from build123d import *
from OCP.BRepFilletAPI import BRepFilletAPI_MakeChamfer

# Parameters (mm, degrees)
BOSS_EXTRUDE1_DEPTH    = 694
SKETCH3_W              = 110
SKETCH3_H              = 70.171613021
CUT_EXTRUDE1_DEPTH     = 145
M10_TAPPED_HOLE2_D     = 8.5
M10_TAPPED_HOLE2_DEPTH = 24.5
M10_TAPPED_HOLE2_TIP   = 2.553657631
BOSS_EXTRUDE2_START    = 44
BOSS_EXTRUDE2_DEPTH    = 44
BOSS_EXTRUDE3_DEPTH    = 44
CUT_EXTRUDE3_DEPTH     = 100
CHAMFER1_SIZE          = 10
CHAMFER1_SIZE2         = 11.749570117
M6_TAPPED_HOLE1_D      = 5
M6_TAPPED_HOLE1_DEPTH  = 15
M6_TAPPED_HOLE1_TIP    = 1.502151548


with BuildPart() as part:
    # Sketch1 → Boss-Extrude1 (new body)
    with BuildSketch(Plane.XY):
        with BuildLine():
            Line((0, 0), (0, -100))
            Line((0, -100), (50, -100))
            Line((50, -100), (50, -98.925311188))
            ThreePointArc((50, -98.925311188), (48.896193111, -95.973045557), (46.126278954, -94.469104878))
            Line((46.126278954, -94.469104878), (13.317028642, -89.858065454))
            ThreePointArc((13.317028642, -89.858065454), (8.084968568, -87.017288616), (6, -81.440786869))
            Line((6, -81.440786869), (6, -18.559213131))
            ThreePointArc((6, -18.559213131), (8.084968568, -12.982711384), (13.317028642, -10.141934546))
            Line((13.317028642, -10.141934546), (46.126278954, -5.530895122))
            ThreePointArc((46.126278954, -5.530895122), (48.896193111, -4.026954443), (50, -1.074688812))
            Line((50, -1.074688812), (50, 0))
            Line((50, 0), (0, 0))
        make_face()
    extrude(amount=BOSS_EXTRUDE1_DEPTH)

    # Sketch3 → Cut-Extrude1 (cut)
    with BuildSketch(Plane.ZY):
        with Locations((247, -120.085806511)):
            Rectangle(SKETCH3_W, SKETCH3_H)
    extrude(amount=-CUT_EXTRUDE1_DEPTH, mode=Mode.SUBTRACT)

    # M10 Tapped Hole2
    with Locations(Plane(origin=(0, 0, 0), x_dir=(1, 0, 0), z_dir=(0, 1, 0))):
        with Locations((25.782416052, -142), (25.782416052, -82), (25.782416052, -22), (25.782416052, -52), (25.782416052, -552), (25.782416052, -612), (25.782416052, -642), (25.782416052, -672)):
            Hole(M10_TAPPED_HOLE2_D / 2, depth=M10_TAPPED_HOLE2_DEPTH)
            with Locations((0, 0, -(M10_TAPPED_HOLE2_DEPTH + M10_TAPPED_HOLE2_TIP / 2))):  # 118° drill point
                Cone(0, M10_TAPPED_HOLE2_D / 2, M10_TAPPED_HOLE2_TIP, mode=Mode.SUBTRACT)

    # Sketch15 → Boss-Extrude2 (add)
    with BuildSketch(Plane(origin=(0, 0, 0), x_dir=(-1, 0, 0), z_dir=(0, 0, -1)).offset(BOSS_EXTRUDE2_START)):
        with BuildLine():
            Line((0, 0), (-50, 0))
            Line((-50, 0), (-50, -1.074688812))
            ThreePointArc((-50, -1.074688812), (-48.896193111, -4.026954443), (-46.126278954, -5.530895122))
            Line((-46.126278954, -5.530895122), (-13.317028642, -10.141934546))
            ThreePointArc((-13.317028642, -10.141934546), (-8.084968568, -12.982711384), (-6, -18.559213131))
            Line((-6, -18.559213131), (-6, -81.440786869))
            ThreePointArc((-6, -81.440786869), (-8.084968568, -87.017288616), (-13.317028642, -89.858065454))
            Line((-13.317028642, -89.858065454), (-46.126278954, -94.469104878))
            ThreePointArc((-46.126278954, -94.469104878), (-48.896193111, -95.973045557), (-50, -98.925311188))
            Line((-50, -98.925311188), (-50, -100))
            Line((-50, -100), (0, -100))
            Line((0, -100), (0, 0))
        make_face()
    extrude(amount=-BOSS_EXTRUDE2_DEPTH)

    # Sketch17 → Boss-Extrude3 (add)
    with BuildSketch(Plane.XY.offset(694)):
        with BuildLine():
            Line((50, 0), (0, 0))
            Line((0, 0), (0, -100))
            Line((0, -100), (50, -100))
            Line((50, -100), (50, -98.925311188))
            ThreePointArc((50, -98.925311188), (48.896193111, -95.973045557), (46.126278954, -94.469104878))
            Line((46.126278954, -94.469104878), (13.317028642, -89.858065454))
            ThreePointArc((13.317028642, -89.858065454), (8.084968568, -87.017288616), (6, -81.440786869))
            Line((6, -81.440786869), (6, -18.559213131))
            ThreePointArc((6, -18.559213131), (8.084968568, -12.982711384), (13.317028642, -10.141934546))
            Line((13.317028642, -10.141934546), (46.126278954, -5.530895122))
            ThreePointArc((46.126278954, -5.530895122), (48.896193111, -4.026954443), (50, -1.074688812))
            Line((50, -1.074688812), (50, 0))
        make_face()
    extrude(amount=BOSS_EXTRUDE3_DEPTH)

    # Sketch16 → Cut-Extrude3 (cut)
    with BuildSketch(Plane.ZY):
        Polygon((6, -100), (-44, -100), (-44, 0), (6, 0), (6, -4.986479132), (-38, -11.170275859), (-38, -88.829724141), (6, -95.013520868), align=None)
        Polygon((688, -95.013520868), (688, -100), (738, -100), (738, 0), (688, 0), (688, -4.986479132), (732, -11.170275859), (732, -88.829724141), align=None)
    extrude(amount=-CUT_EXTRUDE3_DEPTH, mode=Mode.SUBTRACT)

    # Chamfer1: one chamfer whose edges measure the first distance from different faces: ONE call of the kernel's chamfer builder (chamfer() names one face for all edges)
    chamfer1_edges_1 = [part.edges().sort_by_distance(p)[0] for p in [
        (5.149190275, -11.170275859, 732),
    ]]
    chamfer1_side_1 = [part.faces().sort_by_distance(p)[0] for p in [
        (16.706788041, -7.313969364, 704.560953522),
    ]]
    chamfer1_edges_2 = [part.edges().sort_by_distance(p)[0] for p in [
        (5.149190275, -88.829724141, 732),
    ]]
    chamfer1_side_2 = [part.faces().sort_by_distance(p)[0] for p in [
        (3.160002327, -50, 732),
    ]]
    chamfer1_edges_3 = [part.edges().sort_by_distance(p)[0] for p in [
        (5.149190275, -11.170275859, -38),
    ]]
    chamfer1_side_3 = [part.faces().sort_by_distance(p)[0] for p in [
        (3.160002327, -50, -38),
    ]]
    chamfer1_edges_4 = [part.edges().sort_by_distance(p)[0] for p in [
        (5.149190275, -88.829724141, -38),
    ]]
    chamfer1_side_4 = [part.faces().sort_by_distance(p)[0] for p in [
        (16.706788041, -92.686030636, -10.560953522),
    ]]
    chamfer1 = BRepFilletAPI_MakeChamfer(part.part.solid().wrapped)
    for e in chamfer1_edges_1:
        chamfer1.Add(CHAMFER1_SIZE, CHAMFER1_SIZE2, e.wrapped, chamfer1_side_1[0].wrapped)  # the first distance lies on this face
    for e in chamfer1_edges_2:
        chamfer1.Add(CHAMFER1_SIZE, CHAMFER1_SIZE2, e.wrapped, chamfer1_side_2[0].wrapped)  # the first distance lies on this face
    for e in chamfer1_edges_3:
        chamfer1.Add(CHAMFER1_SIZE, CHAMFER1_SIZE2, e.wrapped, chamfer1_side_3[0].wrapped)  # the first distance lies on this face
    for e in chamfer1_edges_4:
        chamfer1.Add(CHAMFER1_SIZE, CHAMFER1_SIZE2, e.wrapped, chamfer1_side_4[0].wrapped)  # the first distance lies on this face
    add(Compound.cast(chamfer1.Shape()), mode=Mode.REPLACE)

    # M6 Tapped Hole1
    with Locations(Plane.ZY):
        with Locations((334.5, -20), (359.5, -20)):
            Hole(M6_TAPPED_HOLE1_D / 2, depth=M6_TAPPED_HOLE1_DEPTH)
            with Locations((0, 0, -(M6_TAPPED_HOLE1_DEPTH + M6_TAPPED_HOLE1_TIP / 2))):  # 118° drill point
                Cone(0, M6_TAPPED_HOLE1_D / 2, M6_TAPPED_HOLE1_TIP, mode=Mode.SUBTRACT)


solid = part.part
Check sheet for the modelled part. Datum: model origin and axes. Units: mm. A direction names the side the tool comes from. Round coordinates to 2 decimals unless told otherwise and drop trailing zeros. Order: outer loops, then holes, each group sorted by start corner. A loop starts at its lowest first (then second) coordinate and runs counter-clockwise, first axis right, second up. Notation, with made-up numbers: M -9,46 L 42,46 A25 cw 42,77 Z; hole C -19.75,69 d8. An arc over 180 degrees is marked long. One line per item, written item: value. Start each with the question number.
1. Gauge pin test, flat ends, axial feed: P1, Ø5.5, axis at x = 28, y = -99, coming from the -Z side; P2, Ø7.5, axis at x = 25.78, z = 82, coming from the +Y side; P3, Ø6.5, axis at y = -20, z = 359.5, coming from the +X side. Record the tip position at first contact, or that the pin passes through.
2. Scan lines: line 1 along Y through (x, z) = (4, 359); line 2 along Y through (x, z) = (16, 681); line 3 along Z through (x, y) = (4, -20). Record each from-to range of solid material in increasing order.
3. Access from +Z, -Z, +X, -X, +Y, -Y to the whole of each face (thin tool, end or side, straight path). Record for faces 4 (the flat face through (6, -50, 342)), 5 (the flat face through (19, -94, 192)), 6 (the flat face through (18.225, -6.817, 701.021)).
4. Section check C-C on z = 293. Enter the section's corners in (x, y), and give its area (3 significant figures).
5. Release check for a two-part mould opening along Y. For faces 1 (the flat face through (29.951, -92.196, 508.553)), 2 (the flat face through (25, 0, 342)), 3 (the flat face through (0, -49, 342)) record: released by +Y, released by -Y, zero draft, split by the parting line, or undercut.
6. Section check B-B on y = -48. Enter the section's corners in (x, z), and give its area (3 significant figures).
7. Section check A-A on z = 468. Enter the section's corners in (x, y), and give its area (3 significant figures).
Results found:
1. P1: z = 6
1. P2: y = -91.08
1. P3: x = 6.19
2. line 1: -100 to -22.45, -17.55 to 0
2. line 2: -100 to -90.24, -9.76 to 0
2. line 3: -36.83 to 332, 337 to 357, 362 to 729.8
3. face 4: +Z, -Z, +X
3. face 5: +X, -X, -Y
3. face 6: +Z, +X, -X, +Y
4. outline: M 0,-85 L 6.78,-85 A8.5 cw 6,-81.44 L 6,-18.56 A8.5 cw 13.32,-10.14 L 46.13,-5.53 A4.5 ccw 50,-1.07 L 50,0 L 0,0 Z
4. area: 874 mm^2
5. face 1: undercut
5. face 2: released by +Y
5. face 3: zero draft
6. outline: M 0,-38 L 6,-38 L 6,732 L 0,732 Z
6. area: 4,620 mm^2
7. outline: M 0,-100 L 50,-100 L 50,-98.93 A4.5 ccw 46.13,-94.47 L 13.32,-89.86 A8.5 cw 6,-81.44 L 6,-18.56 A8.5 cw 13.32,-10.14 L 46.13,-5.53 A4.5 ccw 50,-1.07 L 50,0 L 0,0 Z
7. area: 1,330 mm^2
